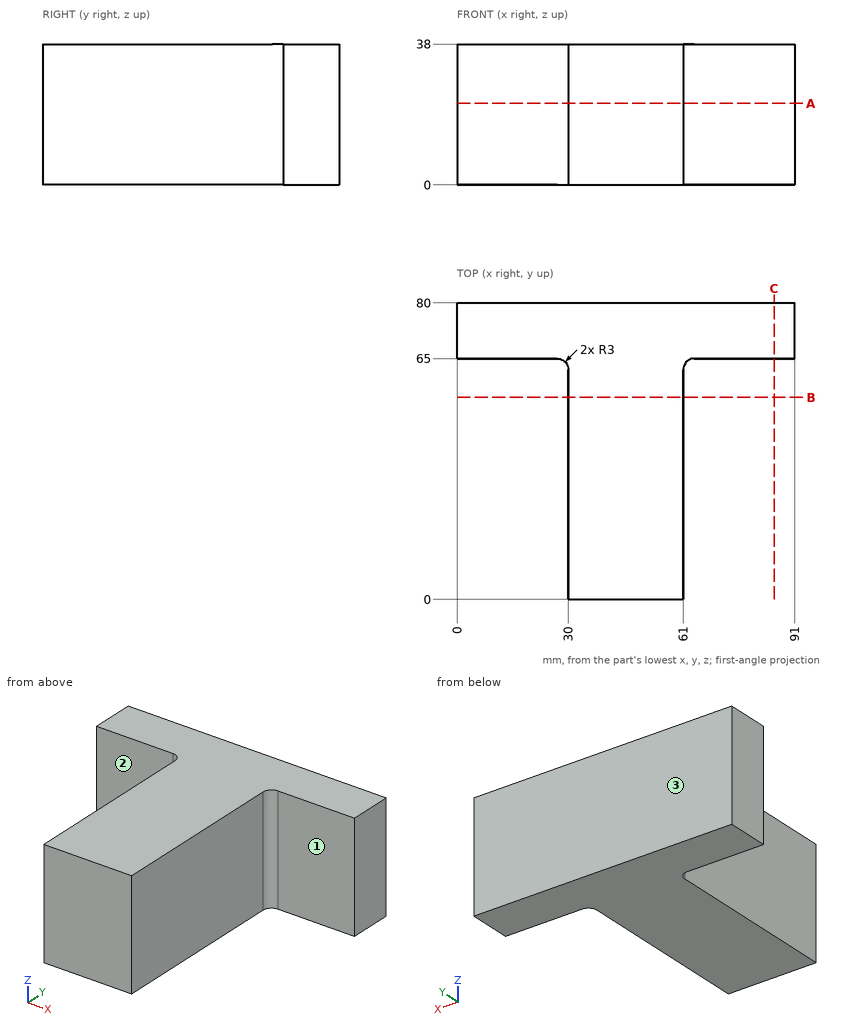
Input: dimensioned drawing with shaded views. Units: mm. Origin: part minimum x, y, z. A direction names the side the tool comes from. Coordinates: 2 decimals unless noted, no trailing zeros. Loops run counter-clockwise (first coordinate to the right, second up) from the corner with the lowest first, then second, coordinate; pieces in that order, holes last. Notation, with made-up numbers: (83, 7) -> (127, 7) arc R23 ccw to (127, 41) -> close; hole circle Ø1 at (1.25, -33.75). An arc over 180 degrees is marked (long way). Use a Markdown table: item, result. Add a question column.
(1) Line query: line 1 along Y through (x, z) = (73, 12.5); line 2 along X through (y, z) = (60, 33); line 3 along X through (y, z) = (63.5, 27). Output: solid intervals per line, ascending.
(2) Pin query (flat end, axial travel): pin 1 Ø12 at (y, z) = (50.5, 14) entering from +X; pin 2 Ø8 at (x, z) = (72.5, 23.5) entering from -Y. Return the tip coordinate at first contact, or that it passes through.
(3) Section query A-A, the plane z = 22. Return loops of the section in (x, y).
(4) Access query for the marked faces 1, 2 and 3. Directions: +Z, -Z, +X, -X, +Y, -Y. A direction counts if a zero-diameter tool reaches every point of the face in a straight line with its end or side. Return the directions, or none.
(5) Section query C-C, the plane x = 85.5. Return loops of the section in (y, z), plus the area to 3 significant figures.
(6) Section query B-B, the plane y = 54.5. Return loops of the section in (x, z), plus the area to 3 significant figures.
Answer:
| question | item | result |
|---|---|---|
| 1 | line 1 | y = 65 to 80 |
| 1 | line 2 | x = 30 to 61 |
| 1 | line 3 | x = 29.6 to 61.4 |
| 2 | pin 1 | stops at x = 61 |
| 2 | pin 2 | stops at y = 65 |
| 3 | outline | (0, 65) -> (27, 65) arc R3 cw to (30, 62) -> (30, 0) -> (61, 0) -> (61, 62) arc R3 cw to (64, 65) -> (91, 65) -> (91, 80) -> (0, 80) -> close |
| 4 | face 1 | +Z, -Z, +X, -Y |
| 4 | face 2 | +Z, -Z, -X, -Y |
| 4 | face 3 | +Z, -Z, +X, -X, +Y |
| 5 | outline | (65, 0) -> (80, 0) -> (80, 38) -> (65, 38) -> close |
| 5 | area | 570 mm^2 |
| 6 | outline | (30, 0) -> (61, 0) -> (61, 38) -> (30, 38) -> close |
| 6 | area | 1,180 mm^2 |
